Read the model definition and answer for the solid it produces. Units are mm, in the model's axes. A direction names the side the tool comes from. Round coordinates to 2 decimals unless told otherwise and drop trailing zeros. Write each loop counter-clockwise with the first axis right and the second up, starting at its lowest first coordinate (ties: lowest second). Pieces come first, ordered by that corner, then holes. Notation, with made-up numbers: (71.5, -26) - (87.5, -26) arc R23 ccw to (87.5, -3) - close; hole circle Ø10 at (-6, 64.5). An arc over 180 degrees is marked (long way). One line per item, written item: value. Start each with the question number.
(1) The mould has two halves that part along Y. Classify faces 3 (the face through (0, -0.6, 7)), 4 (the face through (0.091, 4.499, 7.365)), 5 (the face through (-0.091, -4.499, 7.365)): +Y half, -Y half, draft (parallel to the pull), parting line (faces both ways), or undercut.
(2) Find the intervals of material crossed by L1, parallel to Y at x = 0.5, z = 5.75; L2, parallel to X at y = 3.25, z = 1.5; L3, parallel to Z at x = -4, y = 0, in increasing order.
(3) A cutting plane is placed at C-C, the plane z = 6.5. Determine the outline of the cut face in (x, y) (3 decimals), plus the area to 3 significant figures.
(4) A cutting plane is placed at B-B, the plane x = 0. Determine the outline of the cut face in (y, z) (3 decimals).
(5) A cutting plane is placed at D-D, the plane z = 2. Determine the outline of the cut face in (x, y) (3 decimals).
(6) For faces 1 (the face through (0, 0, 5.5)), 2 (the face through (0, 2, 7.5)), determine the directions among +Z, -Z, +X, -X, +Y, -Y from which every point of the face is accessible in a straight line to the end or side of a thin tool.
(7) Flat-ended cylindrical pins translate along their axes: pin 1 Ø1.5 at (y, z) = (-3.5, 6.5) entering from +X; pin 2 Ø0.6 at (x, z) = (1.5, 7) entering from -Y; pin 3 Ø1 at (y, z) = (-4, 1.5) entering from +X. Find the tip coordinate at first contact, or state that the pin passes through.
(8) A cutting plane is placed at A-A, the plane y = 0. Determine the outline of the cut face in (x, z) (3 decimals), plus the area to 3 significant figures.
from build123d import *

# Parameters (mm, degrees)
SKETCH1_R           = 4.865
BOSS_EXTRUDE1_DEPTH = 7.5
SKETCH2_W           = 12.82033658
SKETCH2_H           = 1.2
CUT_EXTRUDE1_DEPTH  = 2
CHAMFER1_SIZE       = 0.5


with BuildPart() as part:
    # Sketch1 → Boss-Extrude1 (new body)
    with BuildSketch(Plane.XY):
        Circle(SKETCH1_R)
    extrude(amount=BOSS_EXTRUDE1_DEPTH)

    # Sketch2 → Cut-Extrude1 (cut)
    with BuildSketch(Plane.XY.offset(7.5)):
        Rectangle(SKETCH2_W, SKETCH2_H)
    extrude(amount=-CUT_EXTRUDE1_DEPTH, mode=Mode.SUBTRACT)

    # Chamfer1
    chamfer1_edges = [part.edges().sort_by_distance(p)[0] for p in [
        (-4.865, 0, 0),
        (0, 4.865, 7.5),
        (0, -4.865, 7.5),
    ]]
    chamfer(chamfer1_edges, length=CHAMFER1_SIZE)


solid = part.part
Here are the results:
1. face 3: undercut
1. face 4: +Y half
1. face 5: -Y half
2. L1: -4.84 to -0.6, 0.6 to 4.84
2. L2: -3.62 to 3.62
2. L3: 0 to 5.5
3. outline: (-4.828, -0.6) arc R4.865 ccw to (4.828, -0.6) - close; (-4.828, 0.6) - (4.828, 0.6) arc R4.865 ccw to start
3. area: 62.7 mm²
4. outline: (-4.865, 0.5) - (-4.365, 0) - (4.365, 0) - (4.865, 0.5) - (4.865, 7) - (4.365, 7.5) - (0.6, 7.5) - (0.6, 5.5) - (-0.6, 5.5) - (-0.6, 7.5) - (-4.365, 7.5) - (-4.865, 7) - close
5. outline: circle Ø9.73 at (0, 0)
6. face 1: +Z, +X, -X
6. face 2: +Z, +X, -X, +Y, -Y
7. pin 1: x = 4.01
7. pin 2: y = -4.71
7. pin 3: x = 3.38
8. outline: (-4.865, 0.5) - (-4.365, 0) - (4.365, 0) - (4.865, 0.5) - (4.865, 5.5) - (-4.865, 5.5) - close
8. area: 53.3 mm²
